Check sheet for the modelled part. Datum: model origin and axes. Units: mm. A direction names the side the tool comes from. Round coordinates to 2 decimals unless told otherwise and drop trailing zeros. Write each loop counter-clockwise with the first axis right and the second up, starting at its lowest first coordinate (ties: lowest second). Pieces come first, ordered by that corner, then holes. Notation, with made-up numbers: M 85,-23 L 89,-23 A7 ccw 89,-17 Z; hole C 68,79.5 d8. An arc over 180 degrees is marked long. Put each result on its own line as item: value.
```python
from build123d import *

# Parameters (mm, degrees)
EXTRUDE_1_DEPTH              = 15
HOLE_WIZARD_M6_1_D           = 5
HOLE_WIZARD_M6_1_DEPTH       = 15
HOLE_WIZARD_M6_1_CSINK_D     = 6.5
HOLE_WIZARD_M6_1_CSINK_ANGLE = 92
HOLE_WIZARD_M6_1_TIP         = 1.502151548
HOLE_WIZARD_M6_2_D           = 5
HOLE_WIZARD_M6_2_DEPTH       = 15
HOLE_WIZARD_M6_2_CSINK_D     = 6.05
HOLE_WIZARD_M6_2_CSINK_ANGLE = 92
HOLE_WIZARD_M6_2_TIP         = 1.502151548
CHAMFER_1_SIZE               = 0.5
SKETCH_7_W                   = 5.5
SKETCH_7_H                   = 10.083333333
SKETCH_7_W_2                 = 3
SKETCH_7_H_2                 = 20
CUT_EXTRUDE_1_DEPTH          = 127.194294641


with BuildPart() as part:
    # 草图1 → 凸台-拉伸1 (new body)
    with BuildSketch(Plane.XY):
        Polygon((0, 0), (60, 0), (60, 110), align=None)
    extrude(amount=EXTRUDE_1_DEPTH)

    # M6 螺纹孔1
    with Locations(Plane(origin=(0, 0, 0), x_dir=(-1, 0, 0), z_dir=(0, -1, 0))):
        with Locations((-48, -7.5), (-12, -7.5)):
            CounterSinkHole(HOLE_WIZARD_M6_1_D / 2, HOLE_WIZARD_M6_1_CSINK_D / 2, depth=HOLE_WIZARD_M6_1_DEPTH, counter_sink_angle=HOLE_WIZARD_M6_1_CSINK_ANGLE)
            with Locations((0, 0, -(HOLE_WIZARD_M6_1_DEPTH + HOLE_WIZARD_M6_1_TIP / 2))):  # 118° drill point
                Cone(0, HOLE_WIZARD_M6_1_D / 2, HOLE_WIZARD_M6_1_TIP, mode=Mode.SUBTRACT)

    # M6 螺纹孔2
    with Locations(Plane(origin=(60, 0, 0), x_dir=(0, 0, -1), z_dir=(1, 0, 0))):
        with Locations((-7.5, 20), (-7.5, 90)):
            CounterSinkHole(HOLE_WIZARD_M6_2_D / 2, HOLE_WIZARD_M6_2_CSINK_D / 2, depth=HOLE_WIZARD_M6_2_DEPTH, counter_sink_angle=HOLE_WIZARD_M6_2_CSINK_ANGLE)
            with Locations((0, 0, -(HOLE_WIZARD_M6_2_DEPTH + HOLE_WIZARD_M6_2_TIP / 2))):  # 118° drill point
                Cone(0, HOLE_WIZARD_M6_2_D / 2, HOLE_WIZARD_M6_2_TIP, mode=Mode.SUBTRACT)

    # 倒角1
    chamfer_1_edges = [part.edges().sort_by_distance(p)[0] for p in [
        (60, 55, 15),
        (60, 55, 0),
        (30, 55, 15),
        (30, 0, 0),
        (30, 55, 0),
        (30, 0, 15),
    ]]
    chamfer(chamfer_1_edges, length=CHAMFER_1_SIZE)

    # 草图7 → 切除-拉伸1 (cut, through all)
    with BuildSketch(Plane.XY.offset(15)):
        with Locations((57.25, 104.958333334)):
            Rectangle(SKETCH_7_W, SKETCH_7_H)
        with Locations((1.5, 10)):
            Rectangle(SKETCH_7_W_2, SKETCH_7_H_2)
    extrude(amount=-CUT_EXTRUDE_1_DEPTH, mode=Mode.SUBTRACT)


solid = part.part
```
1. Cross-section at A-A (y = 90). Enter the section's corners in (x, z) (3 decimals), then the cut area to 3 significant figures.
Computed values:
outline: M 49.091,0.5 L 49.66,0 L 59.5,0 L 60,0.5 L 60,4.475 L 59.493,5 L 49.091,5 Z; M 49.091,10 L 59.493,10 L 60,10.525 L 60,14.5 L 59.5,15 L 49.66,15 L 49.091,14.5 Z
area: 108 mm2
2. Scan lines: probe 1 along Z at (x, y) = (53.25, 90); probe 2 along Y at (x, z) = (55.5, 7.5); probe 3 along X at (y, z) = (13.5, 7). Record each from-to range of solid material in increasing order.
Computed values:
probe 1: z = 0 to 5, 10 to 15
probe 2: y = 0 to 17.5, 22.5 to 87.5, 92.5 to 99.92
probe 3: x = 7.36 to 9.55, 14.45 to 45.55, 50.45 to 60
3. Depth check by flat-ended pin: pin 1 Ø4 at (y, z) = (48, 9.5) entering from -X; pin 2 Ø4 at (y, z) = (90, 7.5) entering from +X; pin 3 Ø3 at (y, z) = (20, 7.5) entering from +X; pin 4 Ø4.5 at (x, z) = (12, 7.5) entering from +Y (3 decimals). Enter the tip coordinate at first touch or a pass-through.
Computed values:
pin 1: stops at x = 25.09
pin 2: passes through
pin 3: stops at x = 44.4
pin 4: stops at y = 26.125
4. Cross-section at C-C (x = 17). Enter the section's corners in (y, z).
Computed values:
outline: M 0,0.5 L 0.5,0 L 30.12,0 L 31.17,0.5 L 31.17,14.5 L 30.12,15 L 0.5,15 L 0,14.5 Z
5. Cross-section at B-B (y = 11). Enter the section's corners in (x, z), then the cut area to 3 significant figures.
Computed values:
outline: M 6,0.5 L 6.57,0 L 59.5,0 L 60,0.5 L 60,14.5 L 59.5,15 L 6.57,15 L 6,14.5 Z; hole C 12,7.5 d5; hole C 48,7.5 d5
area: 770 mm2
6. Cross-section at D-D (y = 40.5). Enter the section's corners in (x, z), then the cut area to 3 significant figures.
Computed values:
outline: M 22.09,0.5 L 22.66,0 L 59.5,0 L 60,0.5 L 60,14.5 L 59.5,15 L 22.66,15 L 22.09,14.5 Z
area: 568 mm2
7. Access from +Z, -Z, +X, -X, +Y, -Y to the whole of each face (thin tool, end or side, straight path). Record for faces 1 (the cylindrical face through (10, 8, 9)), 2 (the cylindrical face through (52, 22, 9)), 3 (the flat face through (29.11, 53.37, 7.4)).
Computed values:
face 1: -Y
face 2: +X
face 3: +Z, -Z, -X, +Y
8. Release check for a two-part mould opening along Y. For faces 4 (the flat face through (29.18, 52.97, 0.25)), 5 (the conical face through (47.6, 16.24, 7.67)), 6 (the conical face through (43.759, 20.019, 7.934)) record: +Y half, -Y half, draft (parallel to the pull), parting line (faces both ways), or undercut.
Computed values:
face 4: +Y half
face 5: -Y half
face 6: undercut
